Can you work these out from the model? Positions are in its coordinate system, mm. Face numbers are marked on the shaded views. Round coordinates to 2 decimals unless told otherwise and drop trailing zeros. Loops run counter-clockwise (first coordinate to the right, second up) from the corner with the lowest first, then second, coordinate; pieces in that order, holes last. Notation, with made-up numbers: M -14.75,6.25 L 39.25,6.25 A30 ccw 39.25,33.25 Z; hole C 2,12.25 d5. An arc over 180 degrees is marked long. Return JSON: item names as keys, results as strings.
```python
from build123d import *

# Parameters (mm, degrees)
SKETCH1_R           = 5
BOSS_EXTRUDE1_DEPTH = 10


with BuildPart() as part:
    # Sketch1 → Boss-Extrude1 (new body)
    with BuildSketch(Plane.XY):
        with BuildLine():
            Line((-25, 10), (75, 10))
            ThreePointArc((75, 10), (85, 0), (75, -10))
            Line((75, -10), (-25, -10))
            ThreePointArc((-25, -10), (-35, 0), (-25, 10))
        make_face()
        with Locations((75, 0)):
            Circle(SKETCH1_R, mode=Mode.SUBTRACT)
        with Locations((-25, 0)):
            Circle(SKETCH1_R, mode=Mode.SUBTRACT)
    extrude(amount=BOSS_EXTRUDE1_DEPTH)


solid = part.part
```
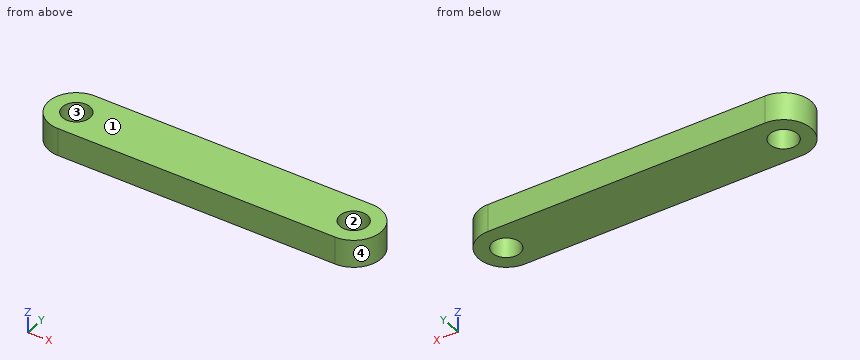
Q1. Suppose I cut it at C-C, the plane y = 7.75. Please give me the cut outline in (x, z), plus the area to 3 significant figures.
Results:
{"outline": "M -31.32,0 L 81.32,0 L 81.32,10 L -31.32,10 Z", "area": "1,130 mm2"}
Q2. If I drill on line 1 along Y through (x, z) = (75, 6); line 2 along X through (y, z) = (-2, 6.25); line 3 along X through (y, z) = (1.25, 6.25), over which ranges is the centre line in solid material (lowest first)?
Results:
{"line 1": "y = -10 to -5, 5 to 10", "line 2": "x = -34.8 to -29.58, -20.42 to 70.42, 79.58 to 84.8", "line 3": "x = -34.92 to -29.84, -20.16 to 70.16, 79.84 to 84.92"}
Q3. I'm going to push flat-ended pins straight in: pin 1 Ø3 at (y, z) = (-7.5, 4.5) entering from -X; pin 2 Ø1 at (y, z) = (2, 7) entering from +X. Where does each tip first touch, or does it pass through?
Results:
{"pin 1": "stops at x = -33", "pin 2": "stops at x = 84.89"}
Q4. Suppose I cut it at B-B, the plane z = 8.5. Please give me the cut outline in (x, y).
Results:
{"outline": "M -25,-10 L 75,-10 A10 ccw 75,10 L -25,10 A10 ccw Z; hole C -25,0 d10; hole C 75,0 d10"}
Q5. Thinking about a two-plate mould opening in Y: for the marked faces 1, 2, 3 and 4, which applies, pulls with the +Y half, pulls with the -Y half, needs draft (parallel to the pull), parting line crosses it, or undercut?
Results:
{"face 1": "needs draft", "face 2": "undercut", "face 3": "undercut", "face 4": "parting line crosses it"}
Q6. Suppose I cut it at A-A, the plane y = 0. Please give me the cut outline in (x, z), plus the area to 3 significant figures.
Results:
{"outline": "M -35,0 L -30,0 L -30,10 L -35,10 Z; M -20,0 L 70,0 L 70,10 L -20,10 Z; M 80,0 L 85,0 L 85,10 L 80,10 Z", "area": "1,000 mm2"}
